```python
from build123d import *

# Parameters (mm, degrees)
SKETCH1_R           = 55
BOSS_EXTRUDE1_DEPTH = 10


with BuildPart() as part:
    # Sketch1 → Boss-Extrude1 (new body)
    with BuildSketch(Plane(origin=(0, 0, 0), x_dir=(0, 0, -1), z_dir=(1, 0, 0))):
        with BuildLine():
            Line((337.625172258, 687.7), (466.146951534, 700.758734438))
            ThreePointArc((466.146951534, 700.758734438), (480.718476107, 698.604521018), (492.508223096, 689.774355121))
            Line((492.508223096, 689.774355121), (823.174539509, 280.80254433))
            ThreePointArc((823.174539509, 280.80254433), (785.648592785, 101.78743459), (617.824738614, 174.518171996))
            ThreePointArc((617.824738614, 174.518171996), (505.411922854, 395.882290886), (317.415259146, 558.042608823))
            ThreePointArc((317.415259146, 558.042608823), (368.029035851, 616.55712727), (337.625172258, 687.7))
        make_face()
        with Locations((731.4, 206.6)):
            Circle(SKETCH1_R, mode=Mode.SUBTRACT)
    extrude(amount=BOSS_EXTRUDE1_DEPTH)


solid = part.part
```
Source: CAD feature listing. Evaluate the final solid. Frame: model axes, mm. Coordinates: 2 decimals unless noted, no trailing zeros. Write each loop counter-clockwise with the first axis right and the second up, starting at its lowest first coordinate (ties: lowest second). Pieces come first, ordered by that corner, then holes. Notation, with made-up numbers: (23.25, -12.5) - (46.25, -12.5) arc R9 cw to (46.25, -7.5) - close; hole circle Ø2 at (45.25, 79). An arc over 180 degrees is marked (long way). Answer as a JSON object with one key per item and string values.
Q1. Section query D-D, the plane y = 513.5. Output: boundary loops of the cut face in (x, z), plus the area to 3 significant figures.
Ans:
{"outline": "(0, -635.03) - (10, -635.03) - (10, -385.33) - (0, -385.33) - close", "area": "2,500 mm2"}
Q2. Draft query along Z for faces 1 (the cylindrical face through (4.93, 152.908, -719.477)), 2 (the flat face through (10, 399, -587)), 3 (the cylindrical face through (4.93, 393.123, -507.561)). Return one class per face: released by +Z, released by -Z, zero draft, split by the parting line, or undercut.
Ans:
{"face 1": "undercut", "face 2": "zero draft", "face 3": "released by +Z"}
Q3. Section query A-A, the plane x = 2.5. Output: boundary loops of the cut face in (y, z), plus the area to 3 significant figures.
Ans:
{"outline": "(174.52, -617.82) arc R118.02 ccw (long way) to (280.8, -823.17) - (689.77, -492.51) arc R30 ccw to (700.76, -466.15) - (687.7, -337.63) arc R73 cw to (558.04, -317.42) arc R642 cw to start; hole circle Ø110 at (206.6, -731.4)", "area": "122,000 mm2"}
Q4. Section query C-C, the plane z = -731.4. Output: boundary loops of the cut face in (x, y), plus the area to 3 significant figures.
Ans:
{"outline": "(0, 88.58) - (10, 88.58) - (10, 151.6) - (0, 151.6) - close; (0, 261.6) - (10, 261.6) - (10, 394.31) - (0, 394.31) - close", "area": "1,960 mm2"}
Q5. Section query B-B, the plane y = 206.6. Output: boundary loops of the cut face in (x, z).
Ans:
{"outline": "(0, -849.42) - (10, -849.42) - (10, -786.4) - (0, -786.4) - close; (0, -676.4) - (10, -676.4) - (10, -607.85) - (0, -607.85) - close"}
Q6. First-contact query: pin 1 Ø3 at (x, y) = (1.5, 552.5) entering from +Z; pin 2 Ø2 at (x, z) = (5.5, -679) entering from -Y; pin 3 Ø1 at (x, z) = (3, -658.5) entering from +Y. Flat tips, straight axial feed; report the tip coordinate or a pass-through.
Ans:
{"pin 1": "stops at z = -324.42", "pin 2": "stops at y = 100.36", "pin 3": "stops at y = 485.09"}
Q7. Material intervals for line 1 (Y direction, x = 2, z = -361); line 2 (Y direction, x = 3, z = -731.4); line 3 (Y direction, x = 5.75, z = -496.5), sorted ascending. Write a range as [from, to].
Ans:
{"line 1": "y = [530.89, 594.77], [660.83, 690.08]", "line 2": "y = [88.58, 151.6], [261.6, 394.31]", "line 3": "y = [407, 684.84]"}
